Part model, mm, in its own coordinate system. Face numbers are marked on the shaded views. Round coordinates to 2 decimals unless told otherwise and drop trailing zeros. Loops run counter-clockwise (first coordinate to the right, second up) from the corner with the lowest first, then second, coordinate; pieces in that order, holes last. Notation, with made-up numbers: (-28, -32) - (23, -32) arc R11 cw to (23, -17) - close; hole circle Ø9 at (-5, -9). An arc over 180 degrees is marked (long way). Put each result on its own line as item: value.
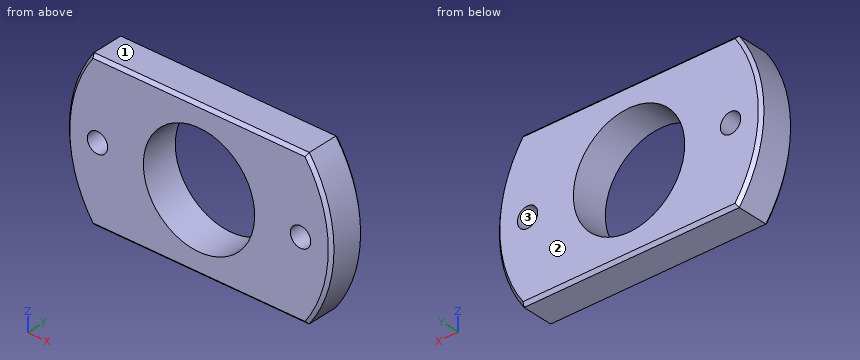
from build123d import *

# Parameters (mm, degrees)
SKETCH_1_R          = 21.5
EXTRUDE_1_DEPTH     = 6
HOLE_WIZARD_M4_1_D  = 3.3
SKETCH_5_W          = 80.188195039
SKETCH_5_H          = 23.165478567
SKETCH_5_W_2        = 146.4427716
SKETCH_5_H_2        = 26.907594335
CUT_EXTRUDE_1_DEPTH = 31.991934435
HOLE_WIZARD_M20_2_D = 18.1
CHAMFER_1_SIZE      = 0.5


with BuildPart() as part:
    # 草图1 → 凸台-拉伸1 (new body)
    with BuildSketch(Plane(origin=(0, 0, 0), x_dir=(1, 0, 0), z_dir=(0, 1, 0))):
        with Locations(Location((0, 0, 0), (0, 0, 270))):
            Circle(SKETCH_1_R)
    extrude(amount=EXTRUDE_1_DEPTH)

    # M4 螺纹孔1 (through all)
    with Locations(Plane(origin=(0, 6, 0), x_dir=(1, 0, 0), z_dir=(0, 1, 0))):
        with Locations((-16.5, 0), (16.5, 0)):
            Hole(HOLE_WIZARD_M4_1_D / 2)

    # 草图5 → 切除-拉伸1 (cut, through all)
    with BuildSketch(Plane(origin=(0, 6, 0), x_dir=(1, 0, 0), z_dir=(0, 1, 0))):
        with Locations((-5.212232678, 24.082739284)):
            Rectangle(SKETCH_5_W, SKETCH_5_H)
        with Locations((21.5, -25.953797168)):
            Rectangle(SKETCH_5_W_2, SKETCH_5_H_2)
    extrude(amount=-CUT_EXTRUDE_1_DEPTH, mode=Mode.SUBTRACT)

    # M20 螺纹孔2 (through all)
    with Locations(Plane(origin=(0, 6, 0), x_dir=(1, 0, 0), z_dir=(0, 1, 0))):
        with Locations((0, 0)):
            Hole(HOLE_WIZARD_M20_2_D / 2)

    # 倒角1
    chamfer_1_edges = [part.edges().sort_by_distance(p)[0] for p in [
        (-21.5, 0, 0),
        (0, 0, -12.5),
        (-21.5, 6, 0),
        (0, 6, -12.5),
        (21.5, 0, 0),
        (0, 0, 12.5),
        (21.5, 6, 0),
        (0, 6, 12.5),
    ]]
    chamfer(chamfer_1_edges, length=CHAMFER_1_SIZE)


solid = part.part
1. Band-saw the part on B-B (y = 4.5). List the corners of the cut face in (x, z), plus the area to 3 significant figures.
A:
outline: (-17.49, -12.5) - (17.49, -12.5) arc R21.5 ccw to (17.49, 12.5) - (-17.49, 12.5) arc R21.5 ccw to start; hole circle Ø3.3 at (-16.5, 0); hole circle Ø18.1 at (0, 0); hole circle Ø3.3 at (16.5, 0)
area: 737 mm²
2. Band-saw the part on D-D (x = 0). List the corners of the cut face in (y, z), plus the area to 3 significant figures.
A:
outline: (0, -12) - (0.5, -12.5) - (5.5, -12.5) - (6, -12) - (6, -9.05) - (0, -9.05) - close; (0, 9.05) - (6, 9.05) - (6, 12) - (5.5, 12.5) - (0.5, 12.5) - (0, 12) - close
area: 40.9 mm²
3. Band-saw the part on A-A (x = -16.5). List the corners of the cut face in (y, z).
A:
outline: (0, -12) - (0.5, -12.5) - (5.5, -12.5) - (6, -12) - (6, -1.65) - (0, -1.65) - close; (0, 1.65) - (6, 1.65) - (6, 12) - (5.5, 12.5) - (0.5, 12.5) - (0, 12) - close
4. Probe line 1 along Z through (x, y) = (0, 4.65); line 2 along X through (y, z) = (1.5, 0.25); line 3 along Z through (x, y) = (-16.5, 3.4). List the from-to ranges inside material, lowest first. Write a range as [from, to].
A:
line 1: z = [-12.5, -9.05], [9.05, 12.5]
line 2: x = [-21.5, -18.13], [-14.87, -9.05], [9.05, 14.87], [18.13, 21.5]
line 3: z = [-12.5, -1.65], [1.65, 12.5]
5. Band-saw the part on C-C (z = 0). List the corners of the cut face in (x, y), plus the area to 3 significant figures.
A:
outline: (-21.5, 0.5) - (-21, 0) - (-18.15, 0) - (-18.15, 6) - (-21, 6) - (-21.5, 5.5) - close; (-14.85, 0) - (-9.05, 0) - (-9.05, 6) - (-14.85, 6) - close; (9.05, 0) - (14.85, 0) - (14.85, 6) - (9.05, 6) - close; (18.15, 0) - (21, 0) - (21.5, 0.5) - (21.5, 5.5) - (21, 6) - (18.15, 6) - close
area: 109 mm²
6. Pin check, flat tip, straight feed: P1, Ø5, axis at x = 7, z = -4.5, coming from the -Y side. Stop position of the tip, or through.
A:
P1: stops at y = 0
7. Two-plate mould, pull along Z, no slides. Class the marked faces 1, 2 and 3: pulls with the +Z half, pulls with the -Z half, needs draft (parallel to the pull), parting line crosses it, or undercut.
A:
face 1: pulls with the +Z half
face 2: needs draft
face 3: undercut
